```python
from build123d import *

# Parameters (mm, degrees)
BOSS_EXTRUDE1_DEPTH = 102


with BuildPart() as part:
    # Sketch1 → Boss-Extrude1 (new body)
    with BuildSketch(Plane.XY):
        with BuildLine():
            Line((0, 0), (-595.74872733, 0))
            ThreePointArc((-595.74872733, 0), (-645.240544835, -7.745145943), (-690, -30.24))
            Line((-690, -30.24), (-683.018424247, -40))
            ThreePointArc((-683.018424247, -40), (-641.574484279, -19.171431429), (-595.74872733, -12))
            Line((-595.74872733, -12), (0, -12))
            Line((0, -12), (0, 0))
        make_face()
    extrude(amount=BOSS_EXTRUDE1_DEPTH)


solid = part.part
```
The listing builds one solid part. Answer for the finished solid, in the listing's coordinates (mm). A direction names the side the tool comes from. Coordinates: 2 decimals unless noted, no trailing zeros. Write each loop counter-clockwise with the first axis right and the second up, starting at its lowest first coordinate (ties: lowest second). Pieces come first, ordered by that corner, then holes.
Q1. Section B-B, the plane x = -120 is taken. Write down the section's boundary in (y, z), then the cut area to 3 significant figures.
Returned:
outline: (-12, 0) - (0, 0) - (0, 102) - (-12, 102) - close
area: 1,220 mm2
Q2. Given P1, Ø10, axis at x = -446, z = 80.5, coming from the -Y side; P2, Ø6, axis at y = -36, z = 27, coming from the -X side; P3, Ø1.5, axis at y = -35, z = 55, coming from the +X side, each flat-ended and moving along its own axis, determine where each tip first touches the part or whether it passes through.
Returned:
P1: stops at y = -12
P2: stops at x = -688.03
P3: stops at x = -674.36
Q3. Section A-A, the plane z = 29 is taken. Write down the section's boundary in (x, y).
Returned:
outline: (-690, -30.24) - (-683.02, -40) arc R150 cw to (-595.75, -12) - (0, -12) - (0, 0) - (-595.75, 0) arc R162 ccw to start
Q4. Find the intervals of material crossed by line 1 along Y through (x, z) = (-76, 9); line 2 along X through (y, z) = (-28, 10); line 3 along Y through (x, z) = (-633, 23.5), in increasing order.
Returned:
line 1: y = -12 to 0
line 2: x = -686.79 to -663.16
line 3: y = -16.7 to -4.34
Q5. Which of the six approach directions +Z, -Z, +X, -X, +Y, -Y give full straight-line access (tool end or side, diameter ignored) to faces 1 (the flat face through (-294, 0, 50)), 2 (the flat face through (-302, -12, 50))?
Returned:
face 1: +Z, -Z, +X, -X, +Y
face 2: +Z, -Z, +X, -Y
Q6. Section C-C, the plane x = -615 is taken. Write down the section's boundary in (y, z), then the cut area to 3 significant figures.
Returned:
outline: (-13.24, 0) - (-1.15, 0) - (-1.15, 102) - (-13.24, 102) - close
area: 1,230 mm2
